```python
from build123d import *

# Parameters (mm, degrees)
BASE_EXTRUDE_DEPTH = 10
SKETCH4_W          = 0.8
SKETCH4_H          = 11.856406461
CHAMFER_2_SIZE     = 1.6
FILLET_2_R         = 0.6


with BuildPart() as part:
    # Sketch1 → Base-Extrude (new body)
    with BuildSketch(Plane(origin=(0, 0, 0), x_dir=(0, 0, -1), z_dir=(1, 0, 0))):
        Polygon((12, 6.92820323), (12, -6.92820323), (0, -13.856406461), (-12, -6.92820323), (-12, 6.92820323), (0, 13.856406461), align=None)
    extrude(amount=BASE_EXTRUDE_DEPTH)

    # Sketch2 → Boss-Revolve1 (revolve)
    with BuildSketch(Plane.XY, mode=Mode.PRIVATE) as boss_revolve1_sk:
        Polygon((0, 0), (170, 0), (170, 6.268), (170, 8), (0, 8), align=None)
    revolve(boss_revolve1_sk.sketch.rotate(Axis((0, 0, 0), (1, 0, 0)), 90), axis=Axis((0, 0, 0), (1, 0, 0)))

    # Sketch3 → Cut-Revolve1 (revolve, cut)
    with BuildSketch(Plane.XY):
        Polygon((0, 12), (3.958548116, 18.856406461), (3.958548116, 23.856406461), (-10, 23.856406461), (-10, 12), align=None)
    revolve(axis=Axis((0, 0, 0), (1, 0, 0)), mode=Mode.SUBTRACT)

    # Sketch5 → Cut-Revolve2 (revolve, cut)
    with BuildSketch(Plane.XY):
        Polygon((10, 12), (6.041451884, 18.856406461), (6.041451884, 23.856406461), (16.041451884, 23.856406461), (16.041451884, 12), align=None)
    revolve(axis=Axis((0, 0, 0), (1, 0, 0)), mode=Mode.SUBTRACT)

    # Sketch4 → Cut-Revolve3 (revolve, cut)
    with BuildSketch(Plane.XY, mode=Mode.PRIVATE) as cut_revolve3_sk:
        with Locations((9.6, 17.928203231)):
            Rectangle(SKETCH4_W, SKETCH4_H)
    revolve(cut_revolve3_sk.sketch.rotate(Axis((0, 0, 0), (1, 0, 0)), 270), axis=Axis((0, 0, 0), (1, 0, 0)), mode=Mode.SUBTRACT)

    # Chamfer 2
    chamfer_2_edges = [part.edges().sort_by_distance(p)[0] for p in [
        (170, 0, -8),
    ]]
    chamfer(chamfer_2_edges, length=CHAMFER_2_SIZE)

    # Fillet 2
    fillet_2_edges = [part.edges().sort_by_distance(p)[0] for p in [
        (10, 0, -8),
    ]]
    fillet(fillet_2_edges, radius=FILLET_2_R)


solid = part.part
```
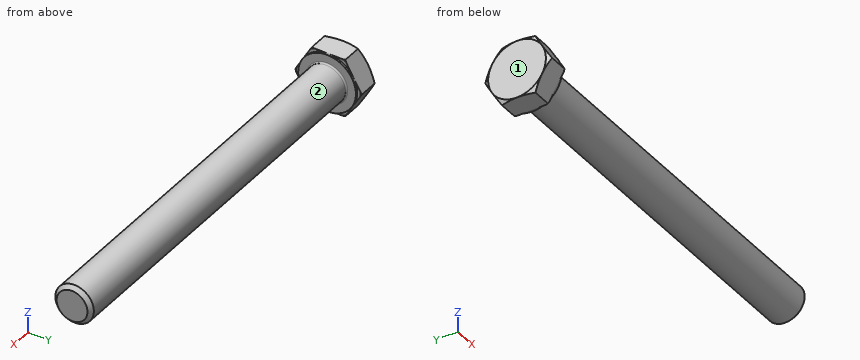
Geometry check sheet. Reference: the model listing, model coordinates, mm. Face numbers are marked on the shaded views. A direction names the side the tool comes from. Coordinates: 2 decimals unless noted, no trailing zeros. Order: outer loops, then holes, each group sorted by start corner. A loop starts at its lowest first (then second) coordinate and runs counter-clockwise, first axis right, second up.
Item 1: Depth check by flat-ended pin: pin 1 (5 mm diameter, centred on x = 55, z = -8, fed in from -Y); pin 2 (3 mm diameter, centred on y = -7.5, z = 9.5, fed in from +X); pin 3 (5 mm diameter, centred on x = 42.5, z = -6.5, fed in from -Y). Enter the tip coordinate at first touch or a pass-through.
Item 2: Tool access check on the marked faces 1 and 2. Record the directions out of +Z, -Z, +X, -X, +Y, -Y that give a thin tool (end or side, any length) a straight path to the whole face; none if there is none.
Item 3: Scan lines: line 1 along X through (y, z) = (8.25, 8.75); line 2 along X through (y, z) = (3.75, -9.5); line 3 along Y through (x, z) = (132, -3). Record each from-to range of solid material in increasing order.
Item 4: Section check A-A (x = 86.5). Enter the section's corners in (y, z), plus the area to 3 significant figures.
Check sheet entries:
1. pin 1: stops at y = -5.81
1. pin 2: stops at x = 10
1. pin 3: stops at y = -6.93
2. face 1: +Z, -Z, -X, +Y, -Y
2. face 2: +X
3. line 1: x = 0.02 to 9.2
3. line 2: x = 0 to 10
3. line 3: y = -7.42 to 7.42
4. outline: circle Ø16 at (0, 0)
4. area: 201 mm2
